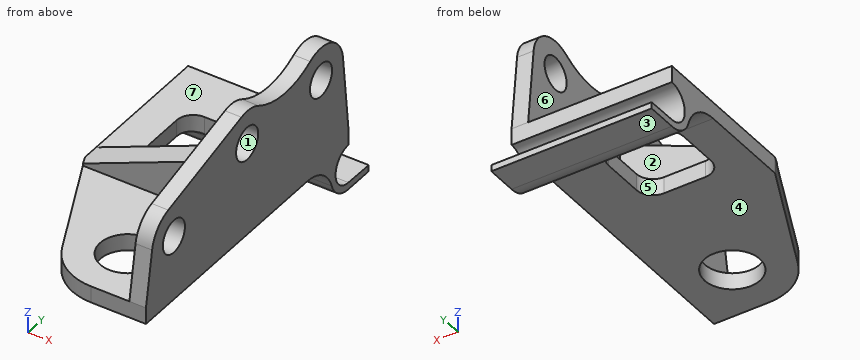
```python
from build123d import *

# Parameters (mm, degrees)
BASE_PLATE_SKETCH_W      = 58
BASE_PLATE_SKETCH_H      = 56
BASE_PLATE_DEPTH         = 6
CHANNEL_WALL_DEPTH       = 58
CHANNEL_GROOVE_CUT_DEPTH = 58
GROOVE_LIP_DEPTH         = 58
SIDE_ARM_DEPTH           = 6
LUG_PLATE_DEPTH          = 6
UPPER_HOLE_SKETCH_R      = 6
UPPER_HOLE_DEPTH         = 6
MIDDLE_HOLE_SKETCH_R     = 10
MIDDLE_HOLE_DEPTH        = 6
GUSSET_DEPTH             = 60
GUSSET_TRIM_CUT_A_DEPTH  = 50
GUSSET_TRIM_CUT_B_DEPTH  = 50
ARM_PROFILE_CUT_DEPTH    = 6
LOWER_HOLE_DEPTH         = 6


with BuildPart() as part:
    # Base Plate Sketch → Base Plate (new body)
    with BuildSketch(Plane.XY):
        with Locations((29, -28)):
            Rectangle(BASE_PLATE_SKETCH_W, BASE_PLATE_SKETCH_H)
    extrude(amount=BASE_PLATE_DEPTH)

    # Channel Wall Sketch → Channel Wall (add)
    with BuildSketch(Plane.ZY):
        with BuildLine():
            Line((0, 0), (-7, 0))
            Line((-7, 0), (-16.5, 0))
            ThreePointArc((-16.5, 0), (-14.652874582, -5.628810766), (-9.829787234, -9.068754281))
            ThreePointArc((-9.829787234, -9.068754281), (-2.722079564, -14.138144724), (0, -22.433234274))
            Line((0, -22.433234274), (0, 0))
        make_face()
    extrude(amount=-CHANNEL_WALL_DEPTH)

    # Channel Groove Sketch → Channel Groove Cut (cut)
    with BuildSketch(Plane.ZY):
        with BuildLine():
            Line((-14, 0), (0, 0))
            ThreePointArc((0, 0), (-7, -7), (-14, 0))
        make_face()
    extrude(amount=-CHANNEL_GROOVE_CUT_DEPTH, mode=Mode.SUBTRACT)

    # Groove Lip Sketch → Groove Lip (add)
    with BuildSketch(Plane.ZY):
        Polygon((-16.5, 0), (-16.5, 11), (-14.179240466, 11), (-14, 0), align=None)
    extrude(amount=-GROOVE_LIP_DEPTH)

    # Side Arm Sketch → Side Arm (add)
    with BuildSketch(Plane.XY.offset(6)):
        with BuildLine():
            Line((58, -109.964049753), (58, -56))
            Line((58, -56), (0, -56))
            Line((0, -56), (19.97833348, -98.476319664))
            ThreePointArc((19.97833348, -98.476319664), (27.35835162, -106.849626412), (38.076434513, -109.964049753))
            Line((38.076434513, -109.964049753), (58, -109.964049753))
        make_face()
    extrude(amount=-SIDE_ARM_DEPTH)

    # Lug Plate Sketch → Lug Plate (add)
    with BuildSketch(Plane(origin=(58, 0, 0), x_dir=(0, 0, -1), z_dir=(1, 0, 0))):
        with BuildLine():
            Line((-6, -109.964049753), (-25.517753411, -106.618685655))
            ThreePointArc((-25.517753411, -106.618685655), (-31.598484509, -103.637669036), (-35.096950284, -97.83917889))
            Line((-35.096950284, -97.83917889), (-45.54096595, -58.069710813))
            ThreePointArc((-45.54096595, -58.069710813), (-45.810409179, -53.300291354), (-44.197856883, -48.803666316))
            ThreePointArc((-44.197856883, -48.803666316), (-40.150792049, -34.831779802), (-43.659207606, -20.715003724))
            ThreePointArc((-43.659207606, -20.715003724), (-43.807215073, -9.350336516), (-34.408466657, -2.959632707))
            Line((-34.408466657, -2.959632707), (-6, 0))
            Line((-6, 0), (-6, -109.964049753))
        make_face()
    extrude(amount=-LUG_PLATE_DEPTH)

    # Upper Hole Sketch → Upper Hole (cut)
    with BuildSketch(Plane.ZY.offset(-52)):
        with Locations((33.165020152, -14.89503554)):
            Circle(UPPER_HOLE_SKETCH_R)
        with Locations((33.934519119, -55.021696385)):
            Circle(UPPER_HOLE_SKETCH_R)
        with Locations((23.490503453, -94.791164461)):
            Circle(UPPER_HOLE_SKETCH_R)
    extrude(amount=-UPPER_HOLE_DEPTH, mode=Mode.SUBTRACT)

    # Middle Hole Sketch → Middle Hole (cut)
    with BuildSketch(Plane.XY.offset(6)):
        with Locations((38.076434513, -89.964049753)):
            Circle(MIDDLE_HOLE_SKETCH_R)
    extrude(amount=-MIDDLE_HOLE_DEPTH, mode=Mode.SUBTRACT)

    # Gusset Sketch → Gusset (add)
    with BuildSketch(Plane(origin=(0, 0, 0), x_dir=(1, 0, 0), z_dir=(0, 1, 0))):
        Polygon((52, -6), (52, -27.93), (0, -6), align=None)
    extrude(amount=-GUSSET_DEPTH)

    # Gusset Trim Sketch A → Gusset Trim Cut A (cut)
    with BuildSketch(Plane(origin=(0, 0, 0), x_dir=(1, 0, 0), z_dir=(0, 1, 0))):
        Polygon((0, -6), (52, -6), (52, -27.93), align=None)
    extrude(amount=-GUSSET_TRIM_CUT_A_DEPTH, mode=Mode.SUBTRACT)

    # Gusset Trim Sketch B → Gusset Trim Cut B (cut)
    with BuildSketch(Plane(origin=(0, 0, 6), x_dir=(-1, 0, 0), z_dir=(0, 0, -1))):
        Polygon((-1.881362005, -60), (0, -56), (0, -60), align=None)
    extrude(amount=-GUSSET_TRIM_CUT_B_DEPTH, mode=Mode.SUBTRACT)

    # Arm Profile Cut Sketch → Arm Profile Cut (cut)
    with BuildSketch(Plane.XY.offset(6)):
        with BuildLine():
            Line((18.5, -46), (33.5, -46))
            ThreePointArc((33.5, -46), (37.742640687, -44.242640687), (39.5, -40))
            Line((39.5, -40), (39.5, -25))
            ThreePointArc((39.5, -25), (37.742640687, -20.757359313), (33.5, -19))
            Line((33.5, -19), (18.5, -19))
            ThreePointArc((18.5, -19), (14.257359313, -20.757359313), (12.5, -25))
            Line((12.5, -25), (12.5, -40))
            ThreePointArc((12.5, -40), (14.257359313, -44.242640687), (18.5, -46))
        make_face()
    extrude(amount=-ARM_PROFILE_CUT_DEPTH, mode=Mode.SUBTRACT)

    # Lower Hole Sketch → Lower Hole (cut)
    with BuildSketch(Plane.XY):
        with BuildLine():
            Line((13.076743256, -22.433234274), (38.923256744, -22.433234274))
            ThreePointArc((38.923256744, -22.433234274), (36.709315008, -19.930453948), (33.5, -19))
            Line((33.5, -19), (18.5, -19))
            ThreePointArc((18.5, -19), (15.290684992, -19.930453948), (13.076743256, -22.433234274))
        make_face()
    extrude(amount=-LOWER_HOLE_DEPTH, mode=Mode.SUBTRACT)


solid = part.part
```
Geometry check sheet. Reference: the model listing, model coordinates, mm. Face numbers are marked on the shaded views. A direction names the side the tool comes from. Coordinates: 2 decimals unless noted, no trailing zeros. Write each loop counter-clockwise with the first axis right and the second up, starting at its lowest first coordinate (ties: lowest second). Pieces come first, ordered by that corner, then holes. Notation, with made-up numbers: M 80.25,38 L 127.25,38 A34 cw 127.25,76 Z; hole C 38,-27 d2. An arc over 180 degrees is marked long. One line per item, written item: value. Start each with the question number.
(1) Sectioned sample at A-A, the plane z = 42. Enter the section's corners in (x, y), and give its area (3 significant figures).
(2) Sectioned sample at D-D, the plane z = 8. Enter the section's corners in (x, y), and give its area (3 significant figures).
(3) Scan lines: line 1 along X through (y, z) = (-103, 13.5); line 2 along Z through (x, y) = (37, -3); line 3 along Z through (x, y) = (32, -69.5). Record each from-to range of solid material in increasing order. Write a range as [from, to].
(4) Release check for a two-part mould opening along Z. For the marked faces 1, 2 and 3 record: released by +Z, released by -Z, zero draft, split by the parting line, or undercut.
(5) Sectioned sample at C-C, the plane x = 54. Enter the section's corners in (y, z) (1 decimal), and give its area (3 significant figures).
(6) Tool access check on the marked faces 4, 5, 6 and 7. Record the directions out of +Z, -Z, +X, -X, +Y, -Y that give a thin tool (end or side, any length) a straight path to the whole face; none if there is none.
(7) Sectioned sample at B-B, the plane y = -41.5. Enter the section's corners in (x, z), and give its area (3 significant figures).
(8) Depth check by flat-ended pin: pin 1 (15 mm diameter, centred on x = 37.5, y = -24, fed in from +Z); pin 2 (2 mm diameter, centred on x = 42, z = -9, fed in from -Y); pin 3 (11 mm diameter, centred on x = 22.5, z = 13, fed in from -Y); pin 4 (14 mm diameter, centred on y = -94.79, z = 23.49, fed in from +X). Enter the tip coordinate at first touch or a pass-through.
Filled sheet:
1. outline: M 52,-71.55 L 58,-71.55 L 58,-44.32 L 52,-44.32 Z; M 52,-24.27 L 58,-24.27 L 58,-6.77 L 52,-6.77 Z
1. area: 268 mm²
2. outline: M 4.74,-60 L 52,-60 L 52,-109.62 L 58,-109.62 L 58,-0.21 L 52,-0.21 L 52,-50 L 4.74,-50 Z
2. area: 1,130 mm²
3. line 1: [52, 58]
3. line 2: [-16.01, -13.32], [-0.68, 6]
3. line 3: [0, 6]
4. face 1: undercut
4. face 2: zero draft
4. face 3: released by -Z
5. outline: M -110,0 L -22.4,0 A14 cw -9.1,-9.8 A9.5 ccw 0,-16.5 L 11,-16.5 L 11,-14.2 L 0,-14 A7 cw 0,0 L 0,6 L -3,34.4 A12 ccw -20.7,43.7 A28 cw -48.8,44.2 A12 ccw -58.1,45.5 L -97.8,35.1 A12 ccw -106.6,25.5 L -110,6 Z; hole C -94.8,23.5 d12; hole C -55,33.9 d12; hole C -14.9,33.2 d12
5. area: 4,130 mm²
6. face 4: -Z, +X, -X, -Y
6. face 5: +Z, -Z
6. face 6: +Z, -X
6. face 7: +Z, -X, +Y
7. outline: M 0,0 L 12.69,0 L 12.69,6 L 0,6 Z; M 39.31,0 L 58,0 L 58,41.09 L 52,41.09 L 52,6 L 39.31,6 Z
7. area: 399 mm²
8. pin 1: z = 6
8. pin 2: y = -9.78
8. pin 3: y = -60
8. pin 4: x = 58
